CAD build for the part. Positions are in the model's coordinates, mm. A direction names the side the tool comes from. Give positions to 0.01 mm unless a question says otherwise; leave off trailing zeros. Write each loop counter-clockwise with the first axis right and the second up, starting at its lowest first coordinate (ties: lowest second). Pieces come first, ordered by that corner, then holes. Notation, with made-up numbers: (10, -22.75) - (33, -22.75) arc R25 cw to (33, 5.25) - close; hole circle Ø2 at (7.25, -18). An arc over 180 degrees is marked (long way). Write item = value, one per line. Start each with the question number.
```python
from build123d import *

# Parameters (mm, degrees)
SKETCH1_R           = 5
BOSS_EXTRUDE1_DEPTH = 500


with BuildPart() as part:
    # Sketch1 → Boss-Extrude1 (new body)
    with BuildSketch(Plane(origin=(0, 0, 0), x_dir=(1, 0, 0), z_dir=(0, 1, 0))):
        Polygon((-6, 20), (-6, 16), (-11.757359313, 16), (-5.757359313, 10), (5.757359313, 10), (11.757359313, 16), (6, 16), (6, 20), (20, 20), (20, 6), (16, 6), (16, 11.757359313), (10, 5.757359313), (10, -5.757359313), (16, -11.757359313), (16, -6), (20, -6), (20, -20), (6, -20), (6, -16), (11.757359313, -16), (5.757359313, -10), (-5.757359313, -10), (-11.757359313, -16), (-6, -16), (-6, -20), (-20, -20), (-20, -6), (-16, -6), (-16, -11.757359313), (-10, -5.757359313), (-10, 5.757359313), (-16, 11.757359313), (-16, 6), (-20, 6), (-20, 20), align=None)
        with Locations(Location((0, 0, 0), (0, 0, 270))):
            Circle(SKETCH1_R, mode=Mode.SUBTRACT)
    extrude(amount=BOSS_EXTRUDE1_DEPTH)


solid = part.part
```
1. Pin check, flat tips, straight feed: pin 1 Ø6 at (y, z) = (298.5, -0.5) entering from +X; pin 2 Ø9 at (x, y) = (1, 371) entering from +Z; pin 3 Ø6 at (x, y) = (-2.5, 301) entering from -Z. Stop position of each tip, or through.
2. Mould opens along X. For faces 4 (the flat face through (0, 246, -10)), 5 (the flat face through (-20, 246, -13)), 6 (the flat face through (-13, 246, 20)) say: +X half, -X half, draft (parallel to the pull), parting line (faces both ways), or undercut.
3. Cut at B-B (z = 0). Give the cut face in (x, y).
4. Tool access for faces 1 (the flat face through (0, 246, 10)), 2 (the flat face through (-10, 246, 0)), 3 (the flat face through (10, 246, 0)): list every direction of +Z, -Z, +X, -X, +Y, -Y with a clear straight run to the whole face (end or side of a thin tool).
5. Cut at A-A (x = 0). Give the cut face in (y, z).
6. Wall check: line 1 along X through (y, z) = (123, -17); line 2 along X through (y, z) = (125, 0); line 3 along Z through (x, y) = (-0.5, 420.5). Give the ranges that are in metal, low to high.
Output:
q1.pin_1 = 10
q1.pin_2 = 10
q1.pin_3 = -10
q2.face_4 = undercut
q2.face_5 = -X half
q2.face_6 = draft
q3.outline = (-10, 0) - (-5, 0) - (-5, 500) - (-10, 500) - close; (5, 0) - (10, 0) - (10, 500) - (5, 500) - close
q4.face_1 = +Z, +Y, -Y
q4.face_2 = -X, +Y, -Y
q4.face_3 = +X, +Y, -Y
q5.outline = (0, -10) - (500, -10) - (500, -5) - (0, -5) - close; (0, 5) - (500, 5) - (500, 10) - (0, 10) - close
q6.line_1 = -20 to -6, 6 to 20
q6.line_2 = -10 to -5, 5 to 10
q6.line_3 = -10 to -4.97, 4.97 to 10
